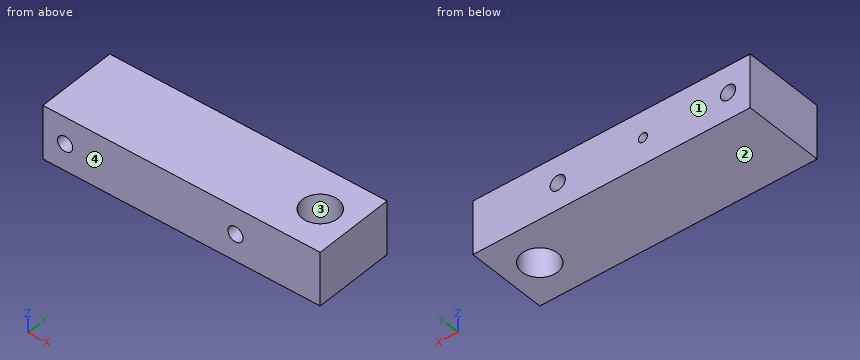
```python
from build123d import *

# Parameters (mm, degrees)
SKETCH_1_W              = 310
SKETCH_1_H              = 90
EXTRUDE_1_DEPTH         = 60
SKETCH_2_R              = 8.5
CUT_EXTRUDE_1_DEPTH     = 90
HOLE_WIZARD_M12_1_D     = 10.2
HOLE_WIZARD_M12_1_DEPTH = 30.25
HOLE_WIZARD_M12_1_TIP   = 3.064389157
SKETCH_6_R              = 20
CUT_EXTRUDE_2_DEPTH     = 60


with BuildPart() as part:
    # 草图1 → 凸台-拉伸1 (new body)
    with BuildSketch(Plane.XY):
        Rectangle(SKETCH_1_W, SKETCH_1_H)
    extrude(amount=EXTRUDE_1_DEPTH)

    # 草图2 → 切除-拉伸1 (cut)
    with BuildSketch(Plane(origin=(0, 45, 0), x_dir=(1, 0, 0), z_dir=(0, 1, 0))):
        with Locations(Location((-130.25, -30, 0), (0, 0, 180))):
            Circle(SKETCH_2_R)
        with Locations(Location((60.25, -30, 0), (0, 0, 180))):
            Circle(SKETCH_2_R)
    extrude(amount=-CUT_EXTRUDE_1_DEPTH, mode=Mode.SUBTRACT)

    # M12 螺纹孔1
    with Locations(Plane(origin=(0, 45, 0), x_dir=(1, 0, 0), z_dir=(0, 1, 0))):
        with Locations((-35, -30)):
            Hole(HOLE_WIZARD_M12_1_D / 2, depth=HOLE_WIZARD_M12_1_DEPTH)
            with Locations((0, 0, -(HOLE_WIZARD_M12_1_DEPTH + HOLE_WIZARD_M12_1_TIP / 2))):  # 118° drill point
                Cone(0, HOLE_WIZARD_M12_1_D / 2, HOLE_WIZARD_M12_1_TIP, mode=Mode.SUBTRACT)

    # 草图6 → 切除-拉伸2 (cut)
    with BuildSketch(Plane(origin=(0, 0, 0), x_dir=(-1, 0, 0), z_dir=(0, 0, -1))):
        with Locations((-117.7, 0)):
            Circle(SKETCH_6_R)
    extrude(amount=-CUT_EXTRUDE_2_DEPTH, mode=Mode.SUBTRACT)


solid = part.part
```
Check sheet for the modelled part. Datum: model origin and axes. Units: mm. Face numbers are marked on the shaded views. Give positions to 0.01 mm unless a question says otherwise; leave off trailing zeros. Order: outer loops, then holes, each group sorted by start corner. A loop starts at its lowest first (then second) coordinate and runs counter-clockwise, first axis right, second up. Notation, with made-up numbers: M 15.5,35.5 L 56.5,35.5 A26 cw 56.5,60.5 Z; hole C -40,-21.75 d1. An arc over 180 degrees is marked long. Answer in a Markdown table with one row per item.
1) Cross-section at A-A, the plane y = 0. Enter the section's corners in (x, z), plus the area to 3 significant figures.
Filled sheet:
| item | result |
|---|---|
| outline | M -155,0 L 97.7,0 L 97.7,60 L -155,60 Z; M 137.7,0 L 155,0 L 155,60 L 137.7,60 Z; hole C -130.25,30 d17; hole C 60.25,30 d17 |
| area | 15,700 mm2 |
2) Release check for a two-part mould opening along Y. For the marked faces 1, 2, 3 and 4 record: +Y half, -Y half, draft (parallel to the pull), parting line (faces both ways), or undercut.
Filled sheet:
| item | result |
|---|---|
| face 1 | +Y half |
| face 2 | draft |
| face 3 | undercut |
| face 4 | -Y half |
3) Cross-section at C-C, the plane y = 36. Enter the section's corners in (x, z).
Filled sheet:
| item | result |
|---|---|
| outline | M -155,0 L 155,0 L 155,60 L -155,60 Z; hole C -130.25,30 d17; hole C -35,30 d10.2; hole C 60.25,30 d17 |
4) Thickness scan on L1, parallel to Z at x = -130, y = -25; L2, parallel to Y at x = 119, z = 12.5; L3, parallel to Z at x = -122.5, y = 28. Record the ranges inside material, lowest first. Write a range as [from, to].
Filled sheet:
| item | result |
|---|---|
| L1 | z = [0, 21.5], [38.5, 60] |
| L2 | y = [-45, -19.96], [19.96, 45] |
| L3 | z = [0, 26.51], [33.49, 60] |
5) Cross-section at D-D, the plane x = 117.7. Enter the section's corners in (y, z), plus the area to 3 significant figures.
Filled sheet:
| item | result |
|---|---|
| outline | M -45,0 L -20,0 L -20,60 L -45,60 Z; M 20,0 L 45,0 L 45,60 L 20,60 Z |
| area | 3,000 mm2 |
6) Cross-section at B-B, the plane x = -130.25. Enter the section's corners in (y, z), plus the area to 3 significant figures.
Filled sheet:
| item | result |
|---|---|
| outline | M -45,0 L 45,0 L 45,21.5 L -45,21.5 Z; M -45,38.5 L 45,38.5 L 45,60 L -45,60 Z |
| area | 3,870 mm2 |
